Read the model definition and answer for the solid it produces. Units are mm, in the model's axes. Face numbers are marked on the shaded views. A direction names the side the tool comes from. Give positions to 0.01 mm unless a question says otherwise; leave off trailing zeros. Loops run counter-clockwise (first coordinate to the right, second up) from the corner with the lowest first, then second, coordinate; pieces in that order, holes last. Notation, with made-up numbers: (10.25, -12.75) - (20.25, -12.75) arc R35 ccw to (20.25, 23.25) - close; hole circle Ø3 at (9, 33.5). An arc over 180 degrees is marked (long way). Use a Markdown table: item, result. Add a question column.
Item 1: A cutting plane is placed at C-C (x = -61.5). Determine the outline of the cut face in (y, z), plus the area to 3 significant figures.
Item 2: For a pull along X with two mould halves and no side action, classify the marked faces 5, 6 and 7 as +X half, -X half, draft (parallel to the pull), parting line (faces both ways), or undercut.
Item 3: Consider probe 1 along Y at (x, z) = (-70, 12.25); probe 2 along X at (y, z) = (-100, 18); probe 3 along Z at (x, y) = (-86, -96.5). Determine where each line is inside the solid, lowest interval first. Write a range as [from, to].
Item 4: Each of these flat-tipped pins is pushed along its axis until it touches: P1, Ø2, axis at y = -48.5, z = 13, coming from the +X side; P2, Ø11.5, axis at y = -73.5, z = 12, coming from the -X side; P3, Ø4, axis at y = -84, z = 24.5, coming from the +X side; P4, Ø6, axis at x = -66.5, z = 6, coming from the -Y side. Where does it stop, or does it pass through?
Item 5: A cutting plane is placed at A-A (z = 16.75). Determine the outline of the cut face in (x, y).
Item 6: A cutting plane is placed at D-D (y = -111). Determine the outline of the cut face in (x, z).
Item 7: A cutting plane is placed at B-B (y = -72). Determine the outline of the cut face in (x, z), plus the area to 3 significant figures.
Item 8: Which of the six approach directions +Z, -Z, +X, -X, +Y, -Y give full straight-line access (tool end or side, diameter ignored) to the marked faces 1, 2, 3 and 4?
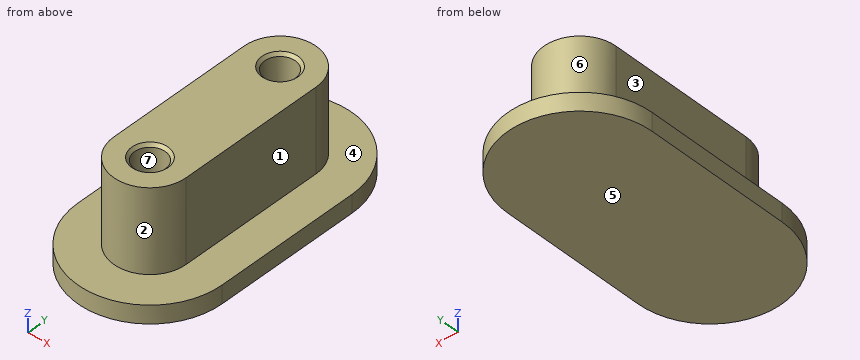
from build123d import *

# Parameters (mm, degrees)
EXTRUDE_1_DEPTH               = 28
EXTRUDE_2_DEPTH               = 5
HOLE_WIZARD_M10_1_D           = 8.5
HOLE_WIZARD_M10_1_DEPTH       = 21.946342369
HOLE_WIZARD_M10_1_CSINK_D     = 10.05
HOLE_WIZARD_M10_1_CSINK_ANGLE = 90
HOLE_WIZARD_M10_1_TIP         = 2.553657631


with BuildPart() as part:
    # 草图1 → 凸台-拉伸1 (new body)
    with BuildSketch(Plane.XY):
        with BuildLine():
            Line((-60, -60), (-60, -100))
            ThreePointArc((-60, -100), (-70, -110), (-80, -100))
            Line((-80, -100), (-80, -60))
            ThreePointArc((-80, -60), (-70, -50), (-60, -60))
        make_face()
    extrude(amount=EXTRUDE_1_DEPTH)

    # 草图2 → 凸台-拉伸2 (add)
    with BuildSketch(Plane.XY):
        with BuildLine():
            Line((-90, -60), (-90, -100))
            ThreePointArc((-90, -100), (-70, -120), (-50, -100))
            Line((-50, -100), (-50, -60))
            ThreePointArc((-50, -60), (-70, -40), (-90, -60))
        make_face()
    extrude(amount=EXTRUDE_2_DEPTH)

    # M10 螺纹孔1
    with Locations(Plane.XY.offset(28)):
        with Locations((-70, -60), (-70, -100)):
            CounterSinkHole(HOLE_WIZARD_M10_1_D / 2, HOLE_WIZARD_M10_1_CSINK_D / 2, depth=HOLE_WIZARD_M10_1_DEPTH, counter_sink_angle=HOLE_WIZARD_M10_1_CSINK_ANGLE)
            with Locations((0, 0, -(HOLE_WIZARD_M10_1_DEPTH + HOLE_WIZARD_M10_1_TIP / 2))):  # 118° drill point
                Cone(0, HOLE_WIZARD_M10_1_D / 2, HOLE_WIZARD_M10_1_TIP, mode=Mode.SUBTRACT)


solid = part.part
Geometry says:
| question | item | result |
|---|---|---|
| 1 | outline | (-118.1, 0) - (-41.9, 0) - (-41.9, 5) - (-54.73, 5) - (-54.73, 28) - (-105.27, 28) - (-105.27, 5) - (-118.1, 5) - close |
| 1 | area | 1,540 mm² |
| 2 | face 5 | draft |
| 2 | face 6 | parting line |
| 2 | face 7 | undercut |
| 3 | probe 1 | [-110, -104.25], [-95.75, -64.25], [-55.75, -50] |
| 3 | probe 2 | [-80, -74.25], [-65.75, -60] |
| 3 | probe 3 | [0, 5] |
| 4 | P1 | through |
| 4 | P2 | x = -80 |
| 4 | P3 | x = -60 |
| 4 | P4 | y = -119.99 |
| 5 | outline | (-80, -100) arc R10 ccw to (-60, -100) - (-60, -60) arc R10 ccw to (-80, -60) - close; hole circle Ø8.5 at (-70, -100); hole circle Ø8.5 at (-70, -60) |
| 6 | outline | (-86.7, 0) - (-53.3, 0) - (-53.3, 5) - (-86.7, 5) - close |
| 7 | outline | (-90, 0) - (-50, 0) - (-50, 5) - (-60, 5) - (-60, 28) - (-80, 28) - (-80, 5) - (-90, 5) - close |
| 7 | area | 660 mm² |
| 8 | face 1 | +Z, +X, +Y, -Y |
| 8 | face 2 | +Z, -Y |
| 8 | face 3 | +Z, -X, +Y, -Y |
| 8 | face 4 | +Z |
